from build123d import *

# Parameters (mm, degrees)
SKETCH1_W               = 470
SKETCH1_H               = 365
BOSS_EXTRUDE1_DEPTH     = 20
CHAMFER1_SIZE           = 20
CUT_EXTRUDE1_DEPTH      = 299.213430281
CUT_EXTRUDE1_DEPTH_BACK = 299.213430281
SKETCH2_R               = 20
CHAMFER2_SIZE           = 20


with BuildPart() as part:
    # Sketch1 → Boss-Extrude1 (new body)
    with BuildSketch(Plane.XY):
        Rectangle(SKETCH1_W, SKETCH1_H)
    extrude(amount=BOSS_EXTRUDE1_DEPTH)

    # Chamfer1
    chamfer1_edges = [part.edges().sort_by_distance(p)[0] for p in [
        (-235, 182.5, 10),
    ]]
    chamfer(chamfer1_edges, length=CHAMFER1_SIZE)

    # Sketch2 → Cut-Extrude1 (cut, two sides: drawn at the far end of the back side and taken through both)
    with BuildSketch(Plane.XY.offset(20).offset(-CUT_EXTRUDE1_DEPTH_BACK)):
        with Locations((-185, 102.5)):
            Circle(SKETCH2_R)
    extrude(amount=CUT_EXTRUDE1_DEPTH + CUT_EXTRUDE1_DEPTH_BACK, mode=Mode.SUBTRACT)

    # Chamfer2
    chamfer2_edges = [part.edges().sort_by_distance(p)[0] for p in [
        (-235, -182.5, 10),
    ]]
    chamfer(chamfer2_edges, length=CHAMFER2_SIZE)


solid = part.part
Verification items for the finished model (mm, model axes). Coordinates: 2 decimals unless noted, no trailing zeros. Order: outer loops, then holes, each group sorted by start corner. A loop starts at its lowest first (then second) coordinate and runs counter-clockwise, first axis right, second up.
Item 1: Section check B-B, the plane x = -185. Enter the section's corners in (y, z).
Filled in:
outline: (-182.5, 0) - (82.5, 0) - (82.5, 20) - (-182.5, 20) - close; (122.5, 0) - (182.5, 0) - (182.5, 20) - (122.5, 20) - close
Item 2: Release check for a two-part mould opening along X. For faces 1 (the face through (-224.9, 172.6, 9.9)), 2 (the face through (7, -182.5, 10)), 3 (the face through (-200.87, 90.33, 9.86)) record: +X half, -X half, draft (parallel to the pull), parting line (faces both ways), or undercut.
Filled in:
face 1: -X half
face 2: draft
face 3: undercut
Item 3: Section check A-A, the plane y = 102.5. Enter the section's corners in (x, z), then the cut area to 3 significant figures.
Filled in:
outline: (-235, 0) - (-205, 0) - (-205, 20) - (-235, 20) - close; (-165, 0) - (235, 0) - (235, 20) - (-165, 20) - close
area: 8,600 mm2
Item 4: Material ranges on L1, parallel to X at y = 102.5, z = 12; L2, parallel to Y at x = -185, z = 15; L3, parallel to Y at x = -187, z = 11.5, recorded low to high.
Filled in:
L1: x = -235 to -205, -165 to 235
L2: y = -182.5 to 82.5, 122.5 to 182.5
L3: y = -182.5 to 82.6, 122.4 to 182.5
